from build123d import *

# Parameters (mm, degrees)
SKETCH_1_W                      = 60
SKETCH_1_H                      = 50
EXTRUDE_1_DEPTH                 = 12
SKETCH_2_W                      = 20
SKETCH_2_H                      = 20
EXTRUDE_2_DEPTH                 = 20
SKETCH_3_R                      = 10.5
CUT_EXTRUDE_1_DEPTH             = 6
CUT_EXTRUDE_2_DEPTH             = 3.5
CUT_EXTRUDE_3_DEPTH             = 3.5
CUT_EXTRUDE_4_DEPTH             = 2.5
CUT_EXTRUDE_5_REACH             = 48.915
SKETCH_8_R                      = 3
CUT_EXTRUDE_5_DIRECTION_2_DEPTH = 47.914816423
SKETCH_9_W                      = 8
SKETCH_9_H                      = 50
CUT_EXTRUDE_6_DEPTH             = 6
CUT_EXTRUDE_START               = -2.5
SKETCH_10_W                     = 14.56297708
SKETCH_10_H                     = 20.2
CUT_EXTRUDE_7_DEPTH             = 12.5
FILLET_1_R                      = 2


with BuildPart() as part:
    # 草图1 → 凸台-拉伸1 (new body)
    with BuildSketch(Plane.XY):
        Rectangle(SKETCH_1_W, SKETCH_1_H)
    extrude(amount=EXTRUDE_1_DEPTH)

    # 草图2 → 凸台-拉伸2 (add)
    with BuildSketch(Plane(origin=(0, 0, 0), x_dir=(-1, 0, 0), z_dir=(0, 0, -1))):
        Rectangle(SKETCH_2_W, SKETCH_2_H)
    extrude(amount=EXTRUDE_2_DEPTH)

    # 草图3 → 切除-拉伸1 (cut)
    with BuildSketch(Plane.XY.offset(12)):
        with Locations((0, -10)):
            Circle(SKETCH_3_R)
    extrude(amount=-CUT_EXTRUDE_1_DEPTH, mode=Mode.SUBTRACT)

    # 草图5 → 切除-拉伸2 (cut)
    with BuildSketch(Plane.XY.offset(12)):
        with BuildLine():
            Line((-18.5, 4.964240044), (-18.5, -1.5))
            ThreePointArc((-18.5, -1.5), (-18.060660172, -2.560660172), (-17, -3))
            Line((-17, -3), (-12.845232579, -3))
            ThreePointArc((-12.845232579, -3), (-12.301125391, -2.897836674), (-11.83113527, -2.605263158))
            ThreePointArc((-11.83113527, -2.605263158), (0, 2), (11.83113527, -2.605263158))
            ThreePointArc((11.83113527, -2.605263158), (12.301125391, -2.897836674), (12.845232579, -3))
            Line((12.845232579, -3), (17, -3))
            ThreePointArc((17, -3), (18.060660172, -2.560660172), (18.5, -1.5))
            Line((18.5, -1.5), (18.5, 4.964240044))
            ThreePointArc((18.5, 4.964240044), (18.412203308, 5.469889941), (18.159090909, 5.916347319))
            ThreePointArc((18.159090909, 5.916347319), (0, 14.5), (-18.159090909, 5.916347319))
            ThreePointArc((-18.159090909, 5.916347319), (-18.412203308, 5.469889941), (-18.5, 4.964240044))
        make_face()
    extrude(amount=-CUT_EXTRUDE_2_DEPTH, mode=Mode.SUBTRACT)

    # 草图6 → 切除-拉伸3 (cut)
    with BuildSketch(Plane.XY.offset(12)):
        with BuildLine():
            Line((-13.389251051, -3), (-14.922616289, -3))
            Line((-14.922616289, -3), (-14.922616289, -25))
            Line((-14.922616289, -25), (14.922616289, -25))
            Line((14.922616289, -25), (14.922616289, -3))
            Line((14.922616289, -3), (13.389251051, -3))
            Line((13.389251051, -3), (13.389251051, -8.470382759))
            Line((13.389251051, -8.470382759), (10.387986864, -8.470382759))
            ThreePointArc((10.387986864, -8.470382759), (10.471959274, -9.233143454), (10.5, -10))
            ThreePointArc((10.5, -10), (-0.766856546, -20.471959274), (-10.387986864, -8.470382759))
            Line((-10.387986864, -8.470382759), (-13.389251051, -8.470382759))
            Line((-13.389251051, -8.470382759), (-13.389251051, -3))
        make_face()
        with BuildLine():
            Line((7.826237921, -3), (-7.826237921, -3))
            ThreePointArc((-7.826237921, -3), (-9.508983543, -5.546997419), (-10.387986864, -8.470382759))
            Line((-10.387986864, -8.470382759), (10.387986864, -8.470382759))
            ThreePointArc((10.387986864, -8.470382759), (9.508983543, -5.546997419), (7.826237921, -3))
        make_face()
        with BuildLine():
            ThreePointArc((7.826237921, -3), (0, 0.5), (-7.826237921, -3))
            Line((-7.826237921, -3), (7.826237921, -3))
        make_face()
        with BuildLine():
            ThreePointArc((-11.83113527, -2.605263158), (-12.301125391, -2.897836674), (-12.845232579, -3))
            Line((-12.845232579, -3), (-7.826237921, -3))
            ThreePointArc((-7.826237921, -3), (0, 0.5), (7.826237921, -3))
            Line((7.826237921, -3), (12.845232579, -3))
            ThreePointArc((12.845232579, -3), (12.301125391, -2.897836674), (11.83113527, -2.605263158))
            ThreePointArc((11.83113527, -2.605263158), (0, 2), (-11.83113527, -2.605263158))
        make_face()
        with BuildLine():
            Line((-12.845232579, -3), (-13.389251051, -3))
            Line((-13.389251051, -3), (-13.389251051, -8.470382759))
            Line((-13.389251051, -8.470382759), (-10.387986864, -8.470382759))
            ThreePointArc((-10.387986864, -8.470382759), (-9.508983543, -5.546997419), (-7.826237921, -3))
            Line((-7.826237921, -3), (-12.845232579, -3))
        make_face()
        with BuildLine():
            Line((12.845232579, -3), (7.826237921, -3))
            ThreePointArc((7.826237921, -3), (9.508983543, -5.546997419), (10.387986864, -8.470382759))
            Line((10.387986864, -8.470382759), (13.389251051, -8.470382759))
            Line((13.389251051, -8.470382759), (13.389251051, -3))
            Line((13.389251051, -3), (12.845232579, -3))
        make_face()
    extrude(amount=-CUT_EXTRUDE_3_DEPTH, mode=Mode.SUBTRACT)

    # 草图7 → 切除-拉伸4 (cut)
    with BuildSketch(Plane.XY.offset(8.5)):
        with BuildLine():
            Line((-18.5, 0.049973913), (-18.5, 0))
            ThreePointArc((-18.5, 0), (-18.060660172, -1.060660172), (-17, -1.5))
            Line((-17, -1.5), (-12.371843032, -1.5))
            ThreePointArc((-12.371843032, -1.5), (-10.253202816, -2.672836244), (-10.122417026, -5.090909091))
            ThreePointArc((-10.122417026, -5.090909091), (0, -21.25), (10.122417026, -5.090909091))
            ThreePointArc((10.122417026, -5.090909091), (10.253202816, -2.672836244), (12.371843032, -1.5))
            Line((12.371843032, -1.5), (17, -1.5))
            ThreePointArc((17, -1.5), (18.060660172, -1.060660172), (18.5, 0))
            Line((18.5, 0), (18.5, 0.049973913))
            ThreePointArc((18.5, 0.049973913), (18.340320328, 0.929121661), (17.881679389, 1.69596379))
            ThreePointArc((17.881679389, 1.69596379), (12.348306903, 6.580233667), (5.752265423, 9.891810345))
            ThreePointArc((5.752265423, 9.891810345), (4.857632257, 10.122405227), (3.93702292, 10.2))
            Line((3.93702292, 10.2), (-3.93702292, 10.2))
            ThreePointArc((-3.93702292, 10.2), (-4.857632257, 10.122405227), (-5.752265423, 9.891810345))
            ThreePointArc((-5.752265423, 9.891810345), (-12.348306903, 6.580233667), (-17.881679389, 1.69596379))
            ThreePointArc((-17.881679389, 1.69596379), (-18.340320328, 0.929121661), (-18.5, 0.049973913))
        make_face()
    extrude(amount=-CUT_EXTRUDE_4_DEPTH, mode=Mode.SUBTRACT)

    # 草图8 → 切除-拉伸5 (cut, up to next)
    with BuildSketch(Plane.XY.offset(6), mode=Mode.PRIVATE) as cut_extrude_5_sk1:
        with Locations(Location((-10, 5, 0), (0, 0, 153.145976086))):
            Circle(SKETCH_8_R)
    cut_extrude_5_tool1 = extrude(cut_extrude_5_sk1.sketch, amount=-CUT_EXTRUDE_5_REACH, mode=Mode.PRIVATE) & part.part
    # 草图8 → 切除-拉伸5 (cut, up to next)
    with BuildSketch(Plane.XY.offset(6), mode=Mode.PRIVATE) as cut_extrude_5_sk2:
        with Locations(Location((10, 5, 0), (0, 0, 90))):
            Circle(SKETCH_8_R)
    cut_extrude_5_tool2 = extrude(cut_extrude_5_sk2.sketch, amount=-CUT_EXTRUDE_5_REACH, mode=Mode.PRIVATE) & part.part
    add(cut_extrude_5_tool1.solids().sort_by_distance((-10, 5, 6))[0], mode=Mode.SUBTRACT)
    add(cut_extrude_5_tool2.solids().sort_by_distance((10, 5, 6))[0], mode=Mode.SUBTRACT)

    # 草图8 → 切除-拉伸5 direction 2 (cut)
    with BuildSketch(Plane.XY.offset(6)):
        with Locations(Location((-10, 5, 0), (0, 0, 153.145976086))):
            Circle(SKETCH_8_R)
        with Locations(Location((10, 5, 0), (0, 0, 90))):
            Circle(SKETCH_8_R)
    extrude(amount=CUT_EXTRUDE_5_DIRECTION_2_DEPTH, mode=Mode.SUBTRACT)

    # 草图9 → 切除-拉伸6 (cut)
    with BuildSketch(Plane.XY.offset(12)):
        with Locations((-26, 0)):
            Rectangle(SKETCH_9_W, SKETCH_9_H)
        with Locations((26, 0)):
            Rectangle(SKETCH_9_W, SKETCH_9_H)
    extrude(amount=-CUT_EXTRUDE_6_DEPTH, mode=Mode.SUBTRACT)

    # 草图10 → 切除-拉伸7 (cut)
    with BuildSketch(Plane.XY.offset(8.5).offset(CUT_EXTRUDE_START)):
        with Locations((-11.21851146, 0.1)):
            Rectangle(SKETCH_10_W, SKETCH_10_H)
    cut_extrude_7 = extrude(amount=CUT_EXTRUDE_7_DEPTH, mode=Mode.SUBTRACT)

    # 镜向2: 切除-拉伸7 across plane
    add(cut_extrude_7.mirror(Plane(origin=(0, 0, 0), x_dir=(0, 0, 1), z_dir=(1, 0, 0))), mode=Mode.SUBTRACT)

    # 圆角1
    fillet_1_edges = [part.edges().sort_by_distance(p)[0] for p in [
        (-18.5, 10.2, 9),
        (-18.5, -10, 9),
        (18.5, -10, 9),
        (18.5, 10.2, 9),
    ]]
    fillet(fillet_1_edges, radius=FILLET_1_R)


solid = part.part
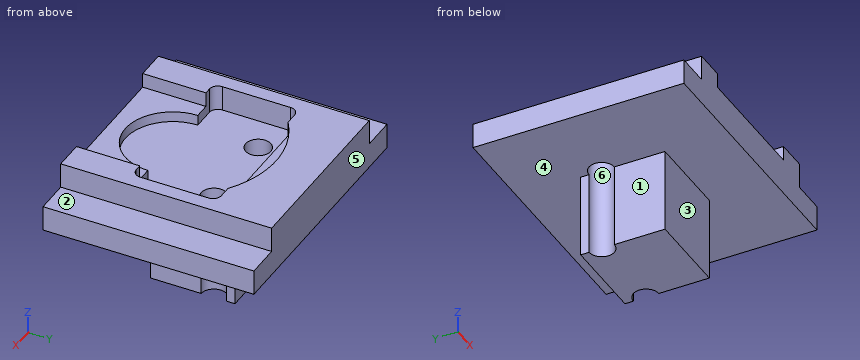
Read the model definition and answer for the solid it produces. Units are mm, in the model's axes. Face numbers are marked on the shaded views. A direction names the side the tool comes from. Give positions to 0.01 mm unless a question says otherwise; leave off trailing zeros. Loops run counter-clockwise (first coordinate to the right, second up) from the corner with the lowest first, then second, coordinate; pieces in that order, holes last. Notation, with made-up numbers: M 12.5,89 L 53.5,89 A28 cw 53.5,118 Z; hole C 31,45 d7. An arc over 180 degrees is marked long. Write each question's results on one line, items separated by ' | '.
1. Given pin 1 (1.5 mm diameter, centred on x = 1.5, z = -14, fed in from +Y); pin 2 (3 mm diameter, centred on y = -0.5, z = -2.5, fed in from -X); pin 3 (3 mm diameter, centred on x = -6, z = 10.5, fed in from -Y), each flat-ended and moving along its own axis, determine where each tip first touches the part or whether it passes through.
Values:
pin 1: stops at y = 10 | pin 2: stops at x = -10 | pin 3: stops at y = 13.27
2. Section B-B on x = 12 is taken. Give the vertices of the cut face in (y, z).
Values:
outline: M -25,0 L 2.76,0 L 2.76,6 L -10,6 L -10,8.5 L -25,8.5 Z; M 7.24,0 L 25,0 L 25,12 L 11.21,12 L 11.21,8.5 L 10.2,8.5 L 10.2,6 L 7.24,6 Z
3. Section D-D on z = -6 is taken. Give the vertices of the cut face in (x, y), plus the area to 3 significant figures.
Values:
outline: M -10,-10 L 10,-10 L 10,2 A3 cw 10,8 L 10,10 L -10,10 L -10,8 A3 cw -10,2 Z | area: 372 mm^2
4. Straight lines are drawn through the part: line 1 (X direction, y = 0.5, z = 10); line 2 (X direction, y = 7, z = 4); line 3 (Z direction, x = 6, y = 11). For each, find the intervals that lie inside material, in ascending order. Write a range as [from, to].
Values:
line 1: x = [-22, -18.5], [18.5, 22] | line 2: x = [-30, -12.24], [-7.76, 7.76], [12.24, 30] | line 3: z = [0, 8.5]
5. A tool of negligible diameter and unlimited length cuts with its end or side. For the marked faces 1, 2 and 3, from which of +Z, -Z, +X, -X, +Y, -Y can it reach the whole face along a straight path? Write none if from no direction.
Values:
face 1: -Z, -X, +Y, -Y | face 2: +Z, +X, +Y, -Y | face 3: -Z, +X, -X, -Y
6. Section A-A on y = 5 is taken. Give the vertices of the cut face in (x, z), plus the area to 3 significant figures.
Values:
outline: M -30,0 L -13,0 L -13,6 L -18.5,6 L -18.5,12 L -22,12 L -22,6 L -30,6 Z; M -7,-20 L 7,-20 L 7,6 L -7,6 Z; M 13,0 L 30,0 L 30,6 L 22,6 L 22,12 L 18.5,12 L 18.5,6 L 13,6 Z | area: 610 mm^2
7. Section C-C on y = -0.5 is taken. Give the vertices of the cut face in (x, z), plus the area to 3 significant figures.
Values:
outline: M -30,0 L -10,0 L -10,-20 L 10,-20 L 10,0 L 30,0 L 30,6 L 22,6 L 22,12 L 18.5,12 L 18.5,6 L -18.5,6 L -18.5,12 L -22,12 L -22,6 L -30,6 Z | area: 802 mm^2
8. The mould has two halves that part along Y. Classify the marked faces 4, 5 and 6: pulls with the +Y half, pulls with the -Y half, needs draft (parallel to the pull), parting line crosses it, or undercut.
Values:
face 4: needs draft | face 5: pulls with the +Y half | face 6: undercut
